Model file for the job. Use its own axes, mm. Face numbers are marked on the shaded views. A direction names the side the tool comes from. Round coordinates to 2 decimals unless told otherwise and drop trailing zeros. Order: outer loops, then holes, each group sorted by start corner. A loop starts at its lowest first (then second) coordinate and runs counter-clockwise, first axis right, second up. Notation, with made-up numbers: M 45,39 L 53,39 A15 ccw 53,43 Z; hole C 36,86.5 d7. An arc over 180 degrees is marked long. Return JSON: item names as keys, results as strings. Group by question number.
Item 1: Slice it at C-C on y = 22.5. Write the cut outline in (x, z).
Item 2: Probe line 1 along X through (y, z) = (23, 9); line 2 along Y through (x, z) = (0, 30.5); line 3 along Y through (x, z) = (22, 4). List the from-to ranges inside material, lowest first.
Item 3: Pull direction X, two halves, no side cores. Call the marked faces 6, 7, 8 and 9: pulls with the +X half, pulls with the -X half, needs draft (parallel to the pull), parting line crosses it, or undercut.
Item 4: Slice it at B-B on y = 0. Write the cut outline in (x, z), then the cut area to 3 significant figures.
Item 5: Which spindle directions (+Z, -Z, +X, -X, +Y, -Y) get a long thin tool onto all of the face, cutting with end or side? Do the marked faces 1, 2, 3, 4 and 5. Say none if no direction does.
Item 6: Slice it at D-D on x = 21. Write the cut outline in (y, z), then the cut area to 3 significant figures.
Item 7: Slice it at A-A on x = 0. Write the cut outline in (y, z).
Item 8: Pin check, flat tips, straight feed: pin 1 Ø2.5 at (y, z) = (-32, 3) entering from +X; pin 2 Ø1.5 at (x, z) = (-34, 6) entering from +Y; pin 3 Ø1.5 at (y, z) = (33, 4.5) entering from -X. Stop position of each tip, or through.
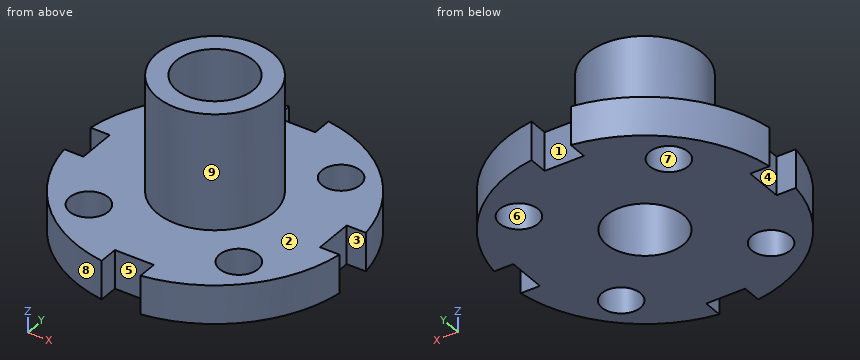
from build123d import *

# Parameters (mm, degrees)
FLANGE_PLATE_DEPTH         = 10
MOUNTING_HOLES_SKETCH_R    = 5
MOUNTING_HOLES_4X_10_DEPTH = 10
HUB_SKETCH_R               = 15
HUB_30_DEPTH               = 30
HUB_BORE_SKETCH_R          = 10
HUB_BORE_20_DEPTH          = 30
FLANGE_BORE_SKETCH_R       = 10
FLANGE_BORE_20_DEPTH       = 30


with BuildPart() as part:
    # Flange Profile Sketch → Flange Plate (new body)
    with BuildSketch(Plane.XY):
        with BuildLine():
            Line((0, 30.693136595), (5.099019514, 30.693136595))
            Line((5.099019514, 30.693136595), (5.099019514, 35.693136595))
            ThreePointArc((5.099019514, 35.693136595), (25.513031554, 25.477150958), (35.700277365, 5.048781643))
            Line((35.700277365, 5.048781643), (30.700277365, 5.048781643))
            Line((30.700277365, 5.048781643), (30.700277365, 0))
            Line((30.700277365, 0), (30.700277365, -5.048781643))
            Line((30.700277365, -5.048781643), (35.700277365, -5.048781643))
            ThreePointArc((35.700277365, -5.048781643), (25.495097568, -25.495097568), (5.048781643, -35.700277365))
            Line((5.048781643, -35.700277365), (5.048781643, -30.700277365))
            Line((5.048781643, -30.700277365), (0, -30.700277365))
            Line((0, -30.700277365), (-5.048781643, -30.700277365))
            Line((-5.048781643, -30.700277365), (-5.048781643, -35.700277365))
            ThreePointArc((-5.048781643, -35.700277365), (-25.512508471, -25.477674767), (-35.707142143, -5))
            Line((-35.707142143, -5), (-30.707142143, -5))
            Line((-30.707142143, -5), (-30.707142143, 0))
            Line((-30.707142143, 0), (-30.707142143, 5))
            Line((-30.707142143, 5), (-35.707142143, 5))
            ThreePointArc((-35.707142143, 5), (-25.530430192, 25.45971591), (-5.099019514, 35.693136595))
            Line((-5.099019514, 35.693136595), (-5.099019514, 30.693136595))
            Line((-5.099019514, 30.693136595), (0, 30.693136595))
        make_face()
    extrude(amount=FLANGE_PLATE_DEPTH)

    # Mounting Holes Sketch → Mounting Holes 4xØ10 (cut)
    with BuildSketch(Plane.XY.offset(10)):
        with Locations((19.445436483, 19.445436483)):
            Circle(MOUNTING_HOLES_SKETCH_R)
        with Locations((19.445436483, -19.445436483)):
            Circle(MOUNTING_HOLES_SKETCH_R)
        with Locations((-19.445436483, -19.445436483)):
            Circle(MOUNTING_HOLES_SKETCH_R)
        with Locations((-19.445436483, 19.445436483)):
            Circle(MOUNTING_HOLES_SKETCH_R)
    extrude(amount=-MOUNTING_HOLES_4X_10_DEPTH, mode=Mode.SUBTRACT)

    # Hub Sketch → Hub Ø30 (add)
    with BuildSketch(Plane.XY.offset(10)):
        Circle(HUB_SKETCH_R)
    extrude(amount=HUB_30_DEPTH)

    # Hub Bore Sketch → Hub Bore Ø20 (cut)
    with BuildSketch(Plane.XY.offset(40)):
        Circle(HUB_BORE_SKETCH_R)
    extrude(amount=-HUB_BORE_20_DEPTH, mode=Mode.SUBTRACT)

    # Flange Bore Sketch → Flange Bore Ø20 (cut)
    with BuildSketch(Plane.XY.offset(10)):
        Circle(FLANGE_BORE_SKETCH_R)
    extrude(amount=-FLANGE_BORE_20_DEPTH, mode=Mode.SUBTRACT)


solid = part.part
Output values:
{
 "1": {"outline": "M -28.17,0 L -23.4,0 L -23.4,10 L -28.17,10 Z; M -15.49,0 L 15.49,0 L 15.49,10 L -15.49,10 Z; M 23.4,0 L 28.17,0 L 28.17,10 L 23.4,10 Z"},
 "2": {"line 1": "-27.77 to -22.96, -15.93 to 15.93, 22.96 to 27.77", "line 2": "-15 to -10, 10 to 15", "line 3": "-28.57 to -23.74, -15.15 to 15.15, 23.74 to 28.57"},
 "3": {"face 6": "undercut", "face 7": "undercut", "face 8": "pulls with the -X half", "face 9": "parting line crosses it"},
 "4": {"outline": "M -30.71,0 L -10,0 L -10,40 L -15,40 L -15,10 L -30.71,10 Z; M 10,0 L 30.7,0 L 30.7,10 L 15,10 L 15,40 L 10,40 Z", "area": "714 mm²"},
 "5": {"face 1": "+Z, -Z, +Y", "face 2": "+Z", "face 3": "+Z, -Z, +X", "face 4": "+Z, -Z, -X", "face 5": "+Z, -Z, -Y"},
 "6": {"outline": "M -29.31,0 L -24.2,0 L -24.2,10 L -29.31,10 Z; M -14.69,0 L 14.69,0 L 14.69,10 L -14.69,10 Z; M 24.2,0 L 29.31,0 L 29.31,10 L 24.2,10 Z", "area": "396 mm²"},
 "7": {"outline": "M -30.7,0 L -10,0 L -10,40 L -15,40 L -15,10 L -30.7,10 Z; M 10,0 L 30.69,0 L 30.69,10 L 15,10 L 15,40 L 10,40 Z"},
 "8": {"pin 1": "x = 18.83", "pin 2": "y = 13.94", "pin 3": "x = -16.12"}
}
